For this review, use the dimensioned drawing (mm, ordinates from the lowest corner) and the shaded views. A direction names the side the tool comes from. Coordinates: 2 decimals unless noted, no trailing zeros. Write each loop counter-clockwise with the first axis right and the second up, starting at its lowest first coordinate (ties: lowest second). Pieces come first, ordered by that corner, then holes. Notation, with made-up numbers: M 4.25,70.25 L 14.25,70.25 A28 cw 14.25,104.25 Z; hole C 78,-11 d8. An arc over 180 degrees is marked long. One line per question, with ' | ' between items.
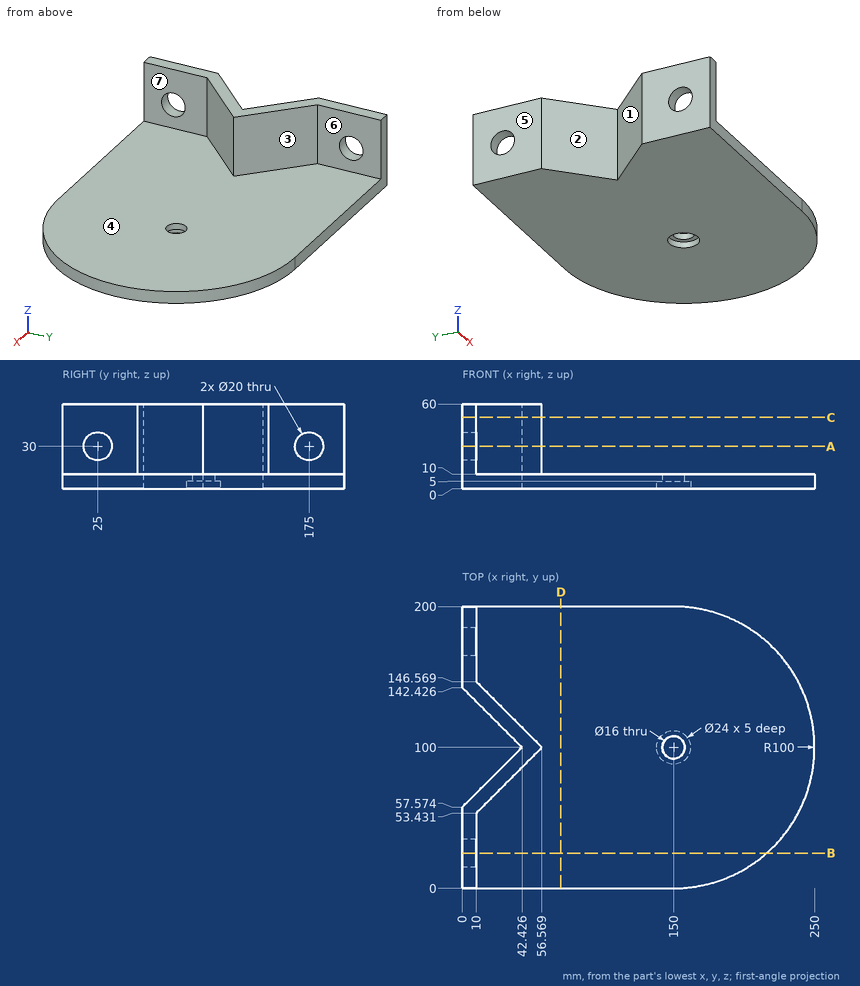
1. Take a section at A-A (z = 30). Write out the cut boundary in (x, y).
Answer sheet:
outline: M 0,0 L 10,0 L 10,15 L 0,15 Z; M 0,35 L 10,35 L 10,53.43 L 56.57,100 L 10,146.57 L 10,165 L 0,165 L 0,142.43 L 42.43,100 L 0,57.57 Z; M 0,185 L 10,185 L 10,200 L 0,200 Z
2. To check wall thickness, follow line 1 along X through (y, z) = (100, 6) (1 decimal); line 2 along Y through (x, z) = (150, 1); line 3 along Y through (x, z) = (150, 7). State the ranges of each line that lie inside material, in increasing order. Write a range as [from, to].
Answer sheet:
line 1: [42.4, 142], [158, 250] | line 2: [0, 88], [112, 200] | line 3: [0, 92], [108, 200]
3. Draft analysis for pull direction Y (two halves, no side actions). For the marked faces 1, 2, 3 and 4, state which applies: pulls with the +Y half, pulls with the -Y half, needs draft (parallel to the pull), parting line crosses it, or undercut.
Answer sheet:
face 1: undercut | face 2: undercut | face 3: pulls with the +Y half | face 4: needs draft
4. Take a section at C-C (z = 50.5). Write out the cut boundary in (x, y), then the cut area to 3 significant figures.
Answer sheet:
outline: M 0,0 L 10,0 L 10,53.43 L 56.57,100 L 10,146.57 L 10,200 L 0,200 L 0,142.43 L 42.43,100 L 0,57.57 Z | area: 2,370 mm^2
5. Insertion check: pin 1 Ø12 at (y, z) = (169.5, 19) entering from +X; pin 2 Ø12 at (y, z) = (25, 30) entering from -X; pin 3 Ø12 at (y, z) = (122.5, 11) entering from -X (1 decimal). Each pin has a flat end and moves straight along its axis. Give the tip position at first contact, or say it passes through.
Answer sheet:
pin 1: x = 10 | pin 2: through | pin 3: x = 13.9
6. Take a section at D-D (x = 70). Write out the cut boundary in (y, z).
Answer sheet:
outline: M 0,0 L 200,0 L 200,10 L 0,10 Z
7. Tool access review of the marked faces 5, 6 and 7: name each direction out of +Z, -Z, +X, -X, +Y, -Y from which nothing blocks a thin tool from reaching the whole face with its end or side.
Answer sheet:
face 5: +Z, -Z, -X, +Y, -Y | face 6: +Z, +X, +Y | face 7: +Z, +X, -Y
8. Take a section at B-B (y = 25). Write out the cut boundary in (x, z).
Answer sheet:
outline: M 0,0 L 216.14,0 L 216.14,10 L 10,10 L 10,20 L 0,20 Z; M 0,40 L 10,40 L 10,60 L 0,60 Z
